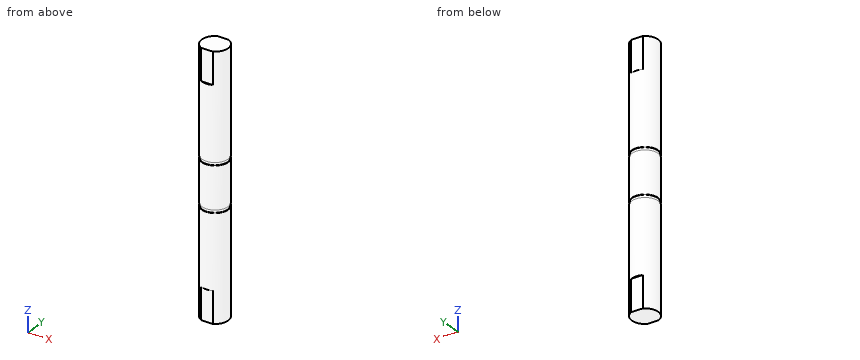
from build123d import *

# Parameters (mm, degrees)
SKETCH_1_R          = 5
EXTRUDE_1_DEPTH     = 49
CUT_EXTRUDE_START   = 1.1
SKETCH_3_R          = 5
SKETCH_3_R_2        = 4.8
CUT_EXTRUDE_2_DEPTH = 1.1
CUT_EXTRUDE_1_DEPTH = 12


with BuildPart() as part:
    # 草图1 → 凸台-拉伸1 (new, symmetric)
    with BuildSketch(Plane.XY):
        Circle(SKETCH_1_R)
    extrude(amount=EXTRUDE_1_DEPTH, both=True)

    # 草图3 → 切除-拉伸2 (cut)
    with BuildSketch(Plane.XY.offset(8).offset(CUT_EXTRUDE_START)):
        Circle(SKETCH_3_R)
        Circle(SKETCH_3_R_2, mode=Mode.SUBTRACT)
    cut_extrude_2 = extrude(amount=-CUT_EXTRUDE_2_DEPTH, mode=Mode.SUBTRACT)

    # 镜向2: 切除-拉伸2 across plane
    add(cut_extrude_2.mirror(Plane.XY), mode=Mode.SUBTRACT)

    # 草图2 → 切除-拉伸1 (cut)
    with BuildSketch(Plane.XY.offset(49)):
        with BuildLine():
            Line((-2.179449472, 4.5), (2.179449472, 4.5))
            ThreePointArc((2.179449472, 4.5), (0, 5), (-2.179449472, 4.5))
        make_face()
        with BuildLine():
            Line((-2.179449472, -4.5), (2.179449472, -4.5))
            ThreePointArc((2.179449472, -4.5), (0, -5), (-2.179449472, -4.5))
        make_face()
    cut_extrude_1 = extrude(amount=-CUT_EXTRUDE_1_DEPTH, mode=Mode.SUBTRACT)

    # 镜向1: 切除-拉伸1 across plane
    add(cut_extrude_1.mirror(Plane.XY), mode=Mode.SUBTRACT)


solid = part.part
Can you work these out from the model? Positions are in its coordinate system, mm. Give positions to 0.01 mm unless a question says otherwise; leave off trailing zeros. Order: outer loops, then holes, each group sorted by start corner. A loop starts at its lowest first (then second) coordinate and runs counter-clockwise, first axis right, second up. Notation, with made-up numbers: M -5,10 L 13,10 A16 ccw 13,17 Z; hole C 84.25,-31.75 d9. An arc over 180 degrees is marked long. Use a Markdown table: item, result. Add a question column.
Item 1: Will these pins go through, and if not, where does the flat tip stop? pin 1 (2 mm diameter, centred on x = 0.5, z = 42.5, fed in from -Y); pin 2 (1 mm diameter, centred on y = 3.5, z = 12, fed in from -X); pin 3 (4 mm diameter, centred on x = 2.5, z = 5.5, fed in from +Y).
Item 2: Suppose I cut it at D-D (z = -20). List the corners of the cut face in (x, y) for me.
Item 3: Suppose I cut it at C-C (y = 1.5). List the corners of the cut face in (x, z) for me, then the cut area to 3 significant figures.
Item 4: Suppose I cut it at B-B (z = 39.5). List the corners of the cut face in (x, y) for me.
Item 5: Suppose I cut it at A-A (x = 0). List the corners of the cut face in (y, z) for me.
Item 6: If I drill on L1, parallel to X at y = 2.25, z = -42.5; L2, parallel to Y at x = -0.25, z = 12.5; L3, parallel to X at y = 3.75, z = -38, over which ranges is the centre line in solid material (lowest first)? Write a range as [from, to].
Answer sheet:
| question | item | result |
|---|---|---|
| 1 | pin 1 | stops at y = -4.5 |
| 1 | pin 2 | stops at x = -4 |
| 1 | pin 3 | stops at y = 4.97 |
| 2 | outline | C 0,0 d10 |
| 3 | outline | M -4.77,-49 L 4.77,-49 L 4.77,-9.1 L 4.56,-9.1 L 4.56,-8 L 4.77,-8 L 4.77,8 L 4.56,8 L 4.56,9.1 L 4.77,9.1 L 4.77,49 L -4.77,49 L -4.77,9.1 L -4.56,9.1 L -4.56,8 L -4.77,8 L -4.77,-8 L -4.56,-8 L -4.56,-9.1 L -4.77,-9.1 Z |
| 3 | area | 934 mm² |
| 4 | outline | M -2.18,-4.5 L 2.18,-4.5 A5 ccw 2.18,4.5 L -2.18,4.5 A5 ccw Z |
| 5 | outline | M -5,-37 L -4.5,-37 L -4.5,-49 L 4.5,-49 L 4.5,-37 L 5,-37 L 5,-9.1 L 4.8,-9.1 L 4.8,-8 L 5,-8 L 5,8 L 4.8,8 L 4.8,9.1 L 5,9.1 L 5,37 L 4.5,37 L 4.5,49 L -4.5,49 L -4.5,37 L -5,37 L -5,9.1 L -4.8,9.1 L -4.8,8 L -5,8 L -5,-8 L -4.8,-8 L -4.8,-9.1 L -5,-9.1 Z |
| 6 | L1 | x = [-4.47, 4.47] |
| 6 | L2 | y = [-4.99, 4.99] |
| 6 | L3 | x = [-3.31, 3.31] |
